Check sheet for the modelled part. Datum: model origin and axes. Units: mm. A direction names the side the tool comes from. Coordinates: 2 decimals unless noted, no trailing zeros. Loops run counter-clockwise (first coordinate to the right, second up) from the corner with the lowest first, then second, coordinate; pieces in that order, holes last. Notation, with made-up numbers: (43, 76.25) -> (51, 76.25) arc R29 cw to (51, 105.25) -> close; hole circle Ø10 at (58.25, -2). An arc over 180 degrees is marked (long way). Use one line per item in the form item = value.
from build123d import *

# Parameters (mm, degrees)
SKETCH_1_W              = 300
SKETCH_1_H              = 320
EXTRUDE_1_DEPTH         = 10
HOLE_WIZARD_M10_1_D     = 8.5
HOLE_WIZARD_M10_1_DEPTH = 15
HOLE_WIZARD_M10_1_TIP   = 2.553657631
SKETCH_7_W              = 90
SKETCH_7_H              = 90
CUT_EXTRUDE_1_DEPTH     = 5
HOLE_WIZARD_M8_1_D      = 6.8
HOLE_WIZARD_M8_1_DEPTH  = 10
HOLE_WIZARD_M8_1_TIP    = 2.042926105
CHAMFER_1_SIZE          = 5


with BuildPart() as part:
    # 草图1 → 凸台-拉伸1 (new, symmetric)
    with BuildSketch(Plane.XY):
        Rectangle(SKETCH_1_W, SKETCH_1_H)
    extrude(amount=EXTRUDE_1_DEPTH, both=True)

    # M10 螺纹孔1
    with Locations(Plane.XY.offset(10)):
        with Locations((50, -20), (-50, -120), (-50, -20), (50, -120)):
            Hole(HOLE_WIZARD_M10_1_D / 2, depth=HOLE_WIZARD_M10_1_DEPTH)
            with Locations((0, 0, -(HOLE_WIZARD_M10_1_DEPTH + HOLE_WIZARD_M10_1_TIP / 2))):  # 118° drill point
                Cone(0, HOLE_WIZARD_M10_1_D / 2, HOLE_WIZARD_M10_1_TIP, mode=Mode.SUBTRACT)

    # 草图7 → 切除-拉伸1 (cut)
    with BuildSketch(Plane.XY.offset(10)):
        with Locations((105, 115)):
            Rectangle(SKETCH_7_W, SKETCH_7_H)
    extrude(amount=-CUT_EXTRUDE_1_DEPTH, mode=Mode.SUBTRACT)

    # M8 螺纹孔1
    with Locations(Plane.XY.offset(5)):
        with Locations((135, 145), (75, 85), (75, 145), (135, 85)):
            Hole(HOLE_WIZARD_M8_1_D / 2, depth=HOLE_WIZARD_M8_1_DEPTH)
            with Locations((0, 0, -(HOLE_WIZARD_M8_1_DEPTH + HOLE_WIZARD_M8_1_TIP / 2))):  # 118° drill point
                Cone(0, HOLE_WIZARD_M8_1_D / 2, HOLE_WIZARD_M8_1_TIP, mode=Mode.SUBTRACT)

    # 倒角1
    chamfer_1_edges = [part.edges().sort_by_distance(p)[0] for p in [
        (150, 160, -2.5),
        (150, -160, 0),
        (-150, -160, 0),
        (-150, 160, 0),
    ]]
    chamfer(chamfer_1_edges, length=CHAMFER_1_SIZE)


solid = part.part
(1) Section check A-A, the plane y = 137.5. Record the boundary of the cut face in (x, z).
Established:
outline = (-150, -10) -> (150, -10) -> (150, 5) -> (60, 5) -> (60, 10) -> (-150, 10) -> close
(2) Tool access check on faces 5 (the flat face through (-2, 2, -10)), 6 (the flat face through (104, 116, 5)), 7 (the cylindrical face through (-46.63, -22.59, 2.39)). Record the directions out of +Z, -Z, +X, -X, +Y, -Y that give a thin tool (end or side, any length) a straight path to the whole face; none if there is none.
Established:
face_5 = -Z, +X, -X, +Y, -Y
face_6 = +Z, +X, +Y
face_7 = +Z
(3) Mould release check, pull along X, two halves, no side actions. Record for faces 1 (the flat face through (-2, 2, 10)), 2 (the flat face through (150, -2, 0)), 3 (the conical face through (49.9, -119.27, -7.11)), 4 (the flat face through (-150, -2, 0)): +X half, -X half, draft (parallel to the pull), parting line (faces both ways), or undercut.
Established:
face_1 = draft
face_2 = +X half
face_3 = undercut
face_4 = -X half
(4) Scan lines: line 1 along Y through (x, z) = (50, -1.75); line 2 along X through (y, z) = (85, -0.75); line 3 along Y through (x, z) = (135, -2). Record each from-to range of solid material in increasing order.
Established:
line_1 = -160 to -124.25, -115.75 to -24.25, -15.75 to 160
line_2 = -150 to 71.6, 78.4 to 131.6, 138.4 to 150
line_3 = -160 to 81.6, 88.4 to 141.6, 148.4 to 160
(5) Go/stop test with flat-tipped pins: P1, Ø4, axis at x = 75, y = 145, coming from the +Z side; P2, Ø4, axis at y = 132.5, z = 8.5, coming from the +X side; P3, Ø2.5, axis at x = 97, z = 6.5, coming from the +Y side. Record where each tip stops, or that it passes through.
Established:
P1 = -5.84
P2 = 60
P3 = 70
